The listing builds one solid part. Answer for the finished solid, in the listing's coordinates (mm). Give positions to 0.01 mm unless a question says otherwise; leave off trailing zeros. Loops run counter-clockwise (first coordinate to the right, second up) from the corner with the lowest first, then second, coordinate; pieces in that order, holes last.
Item 1: Section D-D, the plane x = 80 is taken. Give the vertices of the cut face in (y, z), and give its area (3 significant figures).
Item 2: Section B-B, the plane z = 2.4 is taken. Give the vertices of the cut face in (x, y), and give its area (3 significant figures).
Item 3: Section C-C, the plane x = 60 is taken. Give the vertices of the cut face in (y, z), and give its area (3 significant figures).
Item 4: Section A-A, the plane x = 95 is taken. Give the vertices of the cut face in (y, z), and give its area (3 significant figures).
Item 5: Consider line 1 along X through (y, z) = (20, 2); line 2 along Y through (x, z) = (95, 1.85); line 3 along X through (y, z) = (19.5, 2.2). Determine where each line is inside the solid, lowest interval first.
from build123d import *

# Parameters (mm, degrees)
SKETCH_1_W                   = 100
SKETCH_1_H                   = 25
EXTRUDE_1_DEPTH              = 5
SKETCH_2_R                   = 7.5
SKETCH_2_R_2                 = 4
CUT_EXTRUDE_1_DEPTH          = 104.198837203
HOLE_WIZARD_M3_1_D           = 3.4
HOLE_WIZARD_M3_1_CSINK_D     = 6.72
HOLE_WIZARD_M3_1_CSINK_ANGLE = 90
FILLET_1_R                   = 3
FILLET_2_R                   = 1


with BuildPart() as part:
    # 草图1 → 凸台-拉伸1 (new body)
    with BuildSketch(Plane.XY):
        with Locations((50, 12.5)):
            Rectangle(SKETCH_1_W, SKETCH_1_H)
    extrude(amount=EXTRUDE_1_DEPTH)

    # 草图2 → 切除-拉伸1 (cut, through all)
    with BuildSketch(Plane.XY.offset(5)):
        with Locations((20, 0)):
            Circle(SKETCH_2_R)
        with Locations((40, 0)):
            Circle(SKETCH_2_R)
        with Locations((60, 0)):
            Circle(SKETCH_2_R)
        with Locations((80, 0)):
            Circle(SKETCH_2_R_2)
    extrude(amount=-CUT_EXTRUDE_1_DEPTH, mode=Mode.SUBTRACT)

    # M3 六角凹锥坑螺钉的锥形沉头孔1 (through all)
    with Locations(Plane.XY.offset(5)):
        with Locations((5, 20), (95, 20)):
            CounterSinkHole(HOLE_WIZARD_M3_1_D / 2, HOLE_WIZARD_M3_1_CSINK_D / 2, counter_sink_angle=HOLE_WIZARD_M3_1_CSINK_ANGLE)

    # 圆角1
    fillet_1_edges = [part.edges().sort_by_distance(p)[0] for p in [
        (0, 25, 2.5),
        (100, 25, 2.5),
    ]]
    fillet(fillet_1_edges, radius=FILLET_1_R)

    # 圆角2
    fillet_2_edges = [part.edges().sort_by_distance(p)[0] for p in [
        (100, 11, 5),
        (20, 7.5, 5),
        (20, 7.5, 0),
        (40, 7.5, 5),
        (40, 7.5, 0),
        (60, 7.5, 5),
        (60, 7.5, 0),
        (80, 4, 5),
        (80, 4, 0),
        (100, 11, 0),
        (50, 25, 0),
        (50, 25, 5),
        (0, 11, 0),
        (0.878679656, 24.121320344, 0),
        (99.121320344, 24.121320344, 0),
        (0, 11, 5),
        (0.878679656, 24.121320344, 5),
        (99.121320344, 24.121320344, 5),
    ]]
    fillet(fillet_2_edges, radius=FILLET_2_R)


solid = part.part
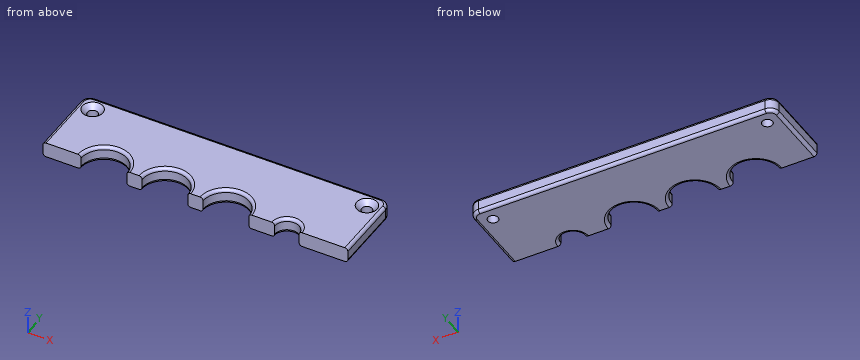
Worked answers:
1. outline: (4, 1) arc R1 ccw to (5, 0) - (24, 0) arc R1 ccw to (25, 1) - (25, 4) arc R1 ccw to (24, 5) - (5, 5) arc R1 ccw to (4, 4) - close
1. area: 104 mm2
2. outline: (0, 0) - (12.5, 0) arc R7.5 cw to (27.5, 0) - (32.5, 0) arc R7.5 cw to (47.5, 0) - (52.5, 0) arc R7.5 cw to (67.5, 0) - (76, 0) arc R4 cw to (84, 0) - (100, 0) - (100, 22) arc R3 ccw to (97, 25) - (3, 25) arc R3 ccw to (0, 22) - close; hole circle Ø3.4 at (5, 20); hole circle Ø3.4 at (95, 20)
2. area: 2,190 mm2
3. outline: (7.5, 1) arc R1 ccw to (8.5, 0) - (24, 0) arc R1 ccw to (25, 1) - (25, 4) arc R1 ccw to (24, 5) - (8.5, 5) arc R1 ccw to (7.5, 4) - close
3. area: 86.6 mm2
4. outline: (0, 0) - (18.3, 0) - (18.3, 3.34) - (16.64, 5) - (0, 5) - close; (21.7, 0) - (24, 0) arc R1 ccw to (25, 1) - (25, 4) arc R1 ccw to (24, 5) - (23.36, 5) - (21.7, 3.34) - close
4. area: 105 mm2
5. line 1: x = 0 to 3.3, 6.7 to 93.3, 96.7 to 100
5. line 2: y = 0 to 18.3, 21.7 to 25
5. line 3: x = 0 to 3.38, 6.62 to 93.38, 96.62 to 100
